The model under review builds one solid part; all positions refer to its coordinate system, in mm. A direction names the side the tool comes from. Coordinates: 2 decimals unless noted, no trailing zeros. Order: outer loops, then holes, each group sorted by start corner. A loop starts at its lowest first (then second) coordinate and runs counter-clockwise, first axis right, second up. Notation, with made-up numbers: M -34.5,29.5 L 20.5,29.5 A27 cw 20.5,53.5 Z; hole C 17.25,-29.75 d7. An arc over 180 degrees is marked long. One line per item, written item: value.
```python
from build123d import *

# Parameters (mm, degrees)
SKETCH1_W           = 660
SKETCH1_H           = 90
SKETCH1_R           = 10
SKETCH1_W_2         = 70
SKETCH1_H_2         = 30
BOSS_EXTRUDE1_DEPTH = 20
BOSS_EXTRUDE2_START = -900
SKETCH2_R           = 10
BOSS_EXTRUDE2_DEPTH = 900
SKETCH3_W           = 903.641141734
SKETCH3_H           = 235.635140662
SKETCH3_W_2         = 650
SKETCH3_H_2         = 80
CUT_EXTRUDE1_DEPTH  = 960.648373103


with BuildPart() as part:
    # Sketch1 → Boss-Extrude1 (new body)
    with BuildSketch(Plane(origin=(0, 0, 0), x_dir=(0, 0, -1), z_dir=(1, 0, 0))):
        Rectangle(SKETCH1_W, SKETCH1_H)
        with Locations((-250, 0)):
            Circle(SKETCH1_R, mode=Mode.SUBTRACT)
        with Locations((250, 0)):
            Circle(SKETCH1_R, mode=Mode.SUBTRACT)
        Rectangle(SKETCH1_W_2, SKETCH1_H_2, mode=Mode.SUBTRACT)
    extrude(amount=BOSS_EXTRUDE1_DEPTH)

    # Sketch2 → Boss-Extrude2 (add)
    with BuildSketch(Plane(origin=(20, 0, 0), x_dir=(0, 0, -1), z_dir=(1, 0, 0)).offset(BOSS_EXTRUDE2_START)):
        with Locations((-250, 0)):
            Circle(SKETCH2_R)
        with Locations((250, 0)):
            Circle(SKETCH2_R)
    extrude(amount=BOSS_EXTRUDE2_DEPTH)

    # Sketch3 → Cut-Extrude1 (cut, through all)
    with BuildSketch(Plane(origin=(20, 0, 0), x_dir=(0, 0, -1), z_dir=(1, 0, 0))):
        Rectangle(SKETCH3_W, SKETCH3_H)
        Rectangle(SKETCH3_W_2, SKETCH3_H_2, mode=Mode.SUBTRACT)
    extrude(amount=-CUT_EXTRUDE1_DEPTH, mode=Mode.SUBTRACT)


solid = part.part
```
(1) Tool access review of faces 5 (the cylindrical face through (-446.16, 3, -259.54)), 6 (the flat face through (10, 0, -35)), 7 (the flat face through (10, -1, -325)): name each direction out of +Z, -Z, +X, -X, +Y, -Y from which nothing blocks a thin tool from reaching the whole face with its end or side.
Geometry results:
face 5: -X
face 6: +X, -X
face 7: -Z, +X, -X, +Y, -Y
(2) We need section D-D, the plane z = -82.5. State the section outline as (x, y) points, plus the area to 3 significant figures.
Geometry results:
outline: M 0,-40 L 20,-40 L 20,40 L 0,40 Z
area: 1,600 mm2
(3) We need section C-C, the plane x = -723. State the section outline as (y, z) points, plus the area to 3 significant figures.
Geometry results:
outline: C 0,-250 d20; C 0,250 d20
area: 628 mm2
(4) Mouldability with a two-part tool opening along Y and no side actions: class faces 1 (the cylindrical face through (-446.16, -3.83, 240.763)), 2 (the flat face through (10, 0, 35)), 3 (the flat face through (10, -15, 0)), 4 (the flat face through (-880, 0, -250)) as +Y half, -Y half, draft (parallel to the pull), parting line (faces both ways), or undercut.
Geometry results:
face 1: parting line
face 2: undercut
face 3: undercut
face 4: draft
(5) For L1, parallel to Z at x = -101, y = 1; L2, parallel to X at y = 2, z = -235.5; L3, parallel to Z at x = -189, y = 7.5, list the stretches that pass through material, from the lowest coordinate up.
Geometry results:
L1: z = -259.95 to -240.05, 240.05 to 259.95
L2: x = 0 to 20
L3: z = -256.61 to -243.39, 243.39 to 256.61
(6) We need section B-B, the plane z = 250. State the section outline as (x, y) points.
Geometry results:
outline: M -880,-10 L 0,-10 L 0,-40 L 20,-40 L 20,40 L 0,40 L 0,10 L -880,10 Z
(7) We need section A-A, the plane y = 0. State the section outline as (x, z) points, plus the area to 3 significant figures.
Geometry results:
outline: M -880,-260 L 0,-260 L 0,-325 L 20,-325 L 20,-35 L 0,-35 L 0,-240 L -880,-240 Z; M -880,240 L 0,240 L 0,35 L 20,35 L 20,325 L 0,325 L 0,260 L -880,260 Z
area: 46,800 mm2
(8) Insertion check: pin 1 Ø4 at (y, z) = (-28, 77.5) entering from -X; pin 2 Ø2 at (x, y) = (-523, -6) entering from -Z. Each pin has a flat end and moves straight along its axis. Give the tip position at first contact, or say it passes through.
Geometry results:
pin 1: stops at x = 0
pin 2: stops at z = -258.66
